```python
from build123d import *

# Parameters (mm, degrees)
SKETCH1_W           = 36
SKETCH1_H           = 18
BOSS_EXTRUDE1_DEPTH = 65
FILLET1_R           = 5
FILLET2_R           = 2


with BuildPart() as part:
    # Sketch1 → Boss-Extrude1 (new body)
    with BuildSketch(Plane.XY):
        Rectangle(SKETCH1_W, SKETCH1_H)
    extrude(amount=BOSS_EXTRUDE1_DEPTH)

    # Fillet1
    fillet1_edges = [part.edges().sort_by_distance(p)[0] for p in [
        (18, -9, 32.5),
        (-18, -9, 32.5),
        (-18, 9, 32.5),
        (18, 9, 32.5),
    ]]
    fillet(fillet1_edges, radius=FILLET1_R)

    # Fillet2
    fillet2_edges = [part.edges().sort_by_distance(p)[0] for p in [
        (0, -9, 0),
        (0, -9, 65),
        (18, 0, 0),
        (-18, 0, 0),
        (0, 9, 0),
        (16.535533906, 7.535533906, 0),
        (16.535533906, -7.535533906, 0),
        (-16.535533906, 7.535533906, 0),
        (-16.535533906, -7.535533906, 0),
        (-18, 0, 65),
        (18, 0, 65),
        (0, 9, 65),
        (16.535533906, 7.535533906, 65),
        (16.535533906, -7.535533906, 65),
        (-16.535533906, 7.535533906, 65),
        (-16.535533906, -7.535533906, 65),
    ]]
    fillet(fillet2_edges, radius=FILLET2_R)


solid = part.part
```
Read the model definition and answer for the solid it produces. Units are mm, in the model's axes. Round coordinates to 2 decimals unless told otherwise and drop trailing zeros. Write each loop counter-clockwise with the first axis right and the second up, starting at its lowest first coordinate (ties: lowest second). Pieces come first, ordered by that corner, then holes. Notation, with made-up numbers: (-10, 21) -> (37, 21) arc R21 ccw to (37, 58) -> close; hole circle Ø1 at (74, 31.25). An arc over 180 degrees is marked (long way). Answer in a Markdown table with one row per item. Add a question column.
1) Find section A-A, the plane z = 47. Determine the outline of the cut face in (x, y), and give its area (3 significant figures).
2) Given P1, Ø2, axis at y = 6.5, z = 37, coming from the +X side, flat-ended and moving along its own axis, determine where the tip first touches the part or whether it passes through.
3) Consider line 1 (X direction, y = -8, z = 38.5); line 2 (Z direction, x = -14.5, y = 7.5); line 3 (X direction, y = 7, z = 12). Determine where each line is inside the solid, lowest interval first.
Findings below:
| question | item | result |
|---|---|---|
| 1 | outline | (-18, -4) arc R5 ccw to (-13, -9) -> (13, -9) arc R5 ccw to (18, -4) -> (18, 4) arc R5 ccw to (13, 9) -> (-13, 9) arc R5 ccw to (-18, 4) -> close |
| 1 | area | 627 mm² |
| 2 | P1 | x = 17.77 |
| 3 | line 1 | -16 to 16 |
| 3 | line 2 | 0.17 to 64.83 |
| 3 | line 3 | -17 to 17 |
